Verification items for the finished model (mm, model axes). Face numbers are marked on the shaded views. A direction names the side the tool comes from. Round coordinates to 2 decimals unless told otherwise and drop trailing zeros. Write each loop counter-clockwise with the first axis right and the second up, starting at its lowest first coordinate (ties: lowest second). Pieces come first, ordered by that corner, then holes. Notation, with made-up numbers: (65, -28) - (98, -28) arc R21 ccw to (98, -14) - close; hole circle Ø9 at (75.5, 66.25). An arc over 180 degrees is marked (long way). Answer as a JSON object with one key per item and string values. Group by question number.
1) Section check A-A (z = 50). Enter the section's corners in (x, y), then the cut area to 3 significant figures.
2) Section check C-C (z = 73.5). Enter the section's corners in (x, y), then the cut area to 3 significant figures.
3) Go/stop test with flat-tipped pins: pin 1 Ø6 at (x, z) = (13.5, 14) entering from +Y; pin 2 Ø23.5 at (y, z) = (-25, 50) entering from +X; pin 3 Ø5 at (y, z) = (-18, 14.5) entering from -X; pin 4 Ø24 at (x, z) = (26.5, 57.5) entering from +Y. Record where each tip stops, or that it passes through.
4) Set-up check for the marked faces 1 and 2: record each of +Z, -Z, +X, -X, +Y, -Y from which the full face is reachable in a straight line by a thin tool's end or side.
5) Thickness scan on line 1 (Y direction, x = 2.5, z = 50); line 2 (X direction, y = -40.5, z = 39); line 3 (Y direction, x = 55, z = 58.5). Record the ranges inside material, lowest first.
6) Section check B-B (y = -25). Enter the section's corners in (x, z).
7) Section check D-D (y = -6.5). Enter the section's corners in (x, z).
```python
from build123d import *

# Parameters (mm, degrees)
BOSS_EXTRUDE1_DEPTH = 100
SKETCH2_R           = 9
CUT_EXTRUDE1_DEPTH  = 100
FILLET1_R           = 5


with BuildPart() as part:
    # Sketch1 → Boss-Extrude1 (new body)
    with BuildSketch(Plane.XY):
        Polygon((0, 0), (0, -80), (60, -80), (60, -73), (7, -73), (7, 0), align=None)
    extrude(amount=BOSS_EXTRUDE1_DEPTH)

    # Sketch2 → Cut-Extrude1 (cut)
    with BuildSketch(Plane(origin=(7, 0, 0), x_dir=(0, 0, -1), z_dir=(1, 0, 0))):
        with Locations((-50, -25)):
            Circle(SKETCH2_R)
    extrude(amount=-CUT_EXTRUDE1_DEPTH, mode=Mode.SUBTRACT)

    # Fillet1
    fillet1_edges = [part.edges().sort_by_distance(p)[0] for p in [
        (7, -73, 50),
    ]]
    fillet(fillet1_edges, radius=FILLET1_R)


solid = part.part
```
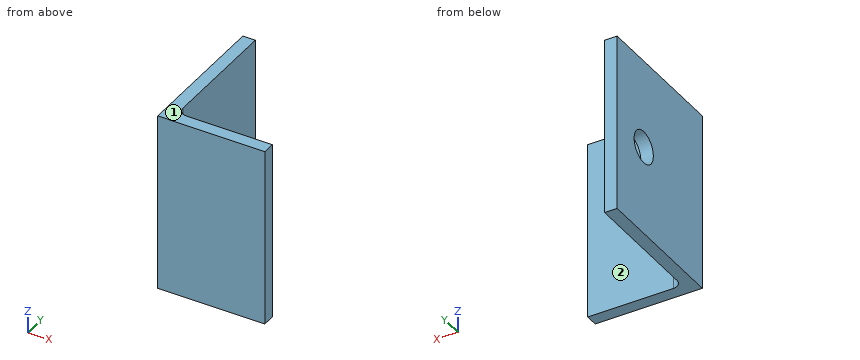
Returned:
{
 "1": {"outline": "(0, -80) - (60, -80) - (60, -73) - (12, -73) arc R5 cw to (7, -68) - (7, -34) - (0, -34) - close; (0, -16) - (7, -16) - (7, 0) - (0, 0) - close", "area": "810 mm2"},
 "2": {"outline": "(0, -80) - (60, -80) - (60, -73) - (12, -73) arc R5 cw to (7, -68) - (7, 0) - (0, 0) - close", "area": "936 mm2"},
 "3": {"pin 1": "y = -72.77", "pin 2": "x = 7", "pin 3": "x = 0", "pin 4": "y = -73"},
 "4": {"face 1": "+Z, +X, -X, +Y, -Y", "face 2": "+Z, -Z, +X, +Y"},
 "5": {"line 1": "-80 to -34, -16 to 0", "line 2": "0 to 7", "line 3": "-80 to -73"},
 "6": {"outline": "(0, 0) - (7, 0) - (7, 41) - (0, 41) - close; (0, 59) - (7, 59) - (7, 100) - (0, 100) - close"},
 "7": {"outline": "(0, 0) - (7, 0) - (7, 100) - (0, 100) - close"}
}
